The listing builds one solid part. Answer for the finished solid, in the listing's coordinates (mm). Coordinates: 2 decimals unless noted, no trailing zeros. Loops run counter-clockwise (first coordinate to the right, second up) from the corner with the lowest first, then second, coordinate; pieces in that order, holes last. Notation, with made-up numbers: (5.25, 29.25) -> (26.25, 29.25) arc R21 ccw to (26.25, 37.25) -> close; hole circle Ø2 at (-12, -22.75). An arc over 180 degrees is marked (long way). Answer in a Markdown table with one row per item.
```python
from build123d import *

# Parameters (mm, degrees)
SKETCH1_W           = 132.8
SKETCH1_H           = 74.7
BOSS_EXTRUDE1_DEPTH = 1
FILLET1_R           = 10


with BuildPart() as part:
    # Sketch1 → Boss-Extrude1 (new body)
    with BuildSketch(Plane.XY):
        Rectangle(SKETCH1_W, SKETCH1_H)
    extrude(amount=BOSS_EXTRUDE1_DEPTH)

    # Fillet1
    fillet1_edges = [part.edges().sort_by_distance(p)[0] for p in [
        (-66.4, -37.35, 0.5),
        (66.4, -37.35, 0.5),
        (66.4, 37.35, 0.5),
        (-66.4, 37.35, 0.5),
    ]]
    fillet(fillet1_edges, radius=FILLET1_R)


solid = part.part
```
Item 1: Find the intervals of material crossed by probe 1 along Y at (x, z) = (57, 0.6); probe 2 along X at (y, z) = (30, 0.3); probe 3 along X at (y, z) = (-31.5, 0.5), in increasing order.
Findings below:
| item | result |
|---|---|
| probe 1 | y = -37.33 to 37.33 |
| probe 2 | x = -66.04 to 66.04 |
| probe 3 | x = -65.5 to 65.5 |
Item 2: A cutting plane is placed at A-A, the plane y = 33.5. Determine the outline of the cut face in (x, z).
Findings below:
| item | result |
|---|---|
| outline | (-64.29, 0) -> (64.29, 0) -> (64.29, 1) -> (-64.29, 1) -> close |
Item 3: A flat-ended cylindrical pin translates along its axis: pin 1 Ø2 at (x, y) = (20, 14.5) entering from -Z. Find the tip coordinate at first contact, or state that the pin passes through.
Findings below:
| item | result |
|---|---|
| pin 1 | stops at z = 0 |
